Geometry check sheet. Reference: the model listing, model coordinates, mm. A direction names the side the tool comes from. Give positions to 0.01 mm unless a question says otherwise; leave off trailing zeros. Order: outer loops, then holes, each group sorted by start corner. A loop starts at its lowest first (then second) coordinate and runs counter-clockwise, first axis right, second up. Notation, with made-up numbers: M 72.25,-25 L 106.25,-25 A20 ccw 106.25,12 Z; hole C 10,-22 d7. An arc over 180 degrees is marked long. Answer as CSV lines item,"result".
from build123d import *

# Parameters (mm, degrees)
SKETCH1_W           = 200
SKETCH1_H           = 116
BOSS_EXTRUDE1_DEPTH = 16


with BuildPart() as part:
    # Sketch1 → Boss-Extrude1 (new body)
    with BuildSketch(Plane.XY):
        with Locations((25, 0)):
            Rectangle(SKETCH1_W, SKETCH1_H)
        with BuildLine():
            Line((0, 30), (50, 30))
            ThreePointArc((50, 30), (80, 0), (50, -30))
            Line((50, -30), (0, -30))
            ThreePointArc((0, -30), (-30, 0), (0, 30))
        make_face(mode=Mode.SUBTRACT)
    extrude(amount=BOSS_EXTRUDE1_DEPTH)


solid = part.part
(1) Section check B-B on z = 11.25. Enter the section's corners in (x, y), then the cut area to 3 significant figures.
The answers:
outline,"M -75,-58 L 125,-58 L 125,58 L -75,58 Z; hole M 0,-30 L 50,-30 A30 ccw 50,30 L 0,30 A30 ccw Z"
area,"17,400 mm2"
(2) Tool access check on faces 4 (the face through (125, -1, 8)), 5 (the face through (79.993, 0.66, 7.888)). Record the directions out of +Z, -Z, +X, -X, +Y, -Y that give a thin tool (end or side, any length) a straight path to the whole face; none if there is none.
The answers:
face 4,"+Z, -Z, +X, +Y, -Y"
face 5,"+Z, -Z"
(3) Material ranges on line 1 (Y direction, x = 10, z = 6); line 2 (X direction, y = -18.5, z = 4.25); line 3 (X direction, y = 7, z = 7), recorded low to high.
The answers:
line 1,"y = -58 to -30, 30 to 58"
line 2,"x = -75 to -23.62, 73.62 to 125"
line 3,"x = -75 to -29.17, 79.17 to 125"
(4) Gauge pin test, flat end, axial feed: P1, Ø1.5, axis at x = 94.5, y = 19.5, coming from the -Z side. Record the tip position at first contact, or that the pin passes through.
The answers:
P1,"stops at z = 0"
(5) Section check A-A on y = 0. Enter the section's corners in (x, z).
The answers:
outline,"M -75,0 L -30,0 L -30,16 L -75,16 Z; M 80,0 L 125,0 L 125,16 L 80,16 Z"
(6) Section check C-C on x = 73.5. Enter the section's corners in (y, z).
The answers:
outline,"M -58,0 L -18.65,0 L -18.65,16 L -58,16 Z; M 18.65,0 L 58,0 L 58,16 L 18.65,16 Z"
(7) Draft check along Y on faces 1 (the face through (24, 58, 8)), 2 (the face through (-29.993, -0.66, 7.888)), 3 (the face through (-75, -1, 8)). Enter one of: +Y half, -Y half, draft (parallel to the pull), parting line (faces both ways), or undercut.
The answers:
face 1,"+Y half"
face 2,"undercut"
face 3,"draft"
